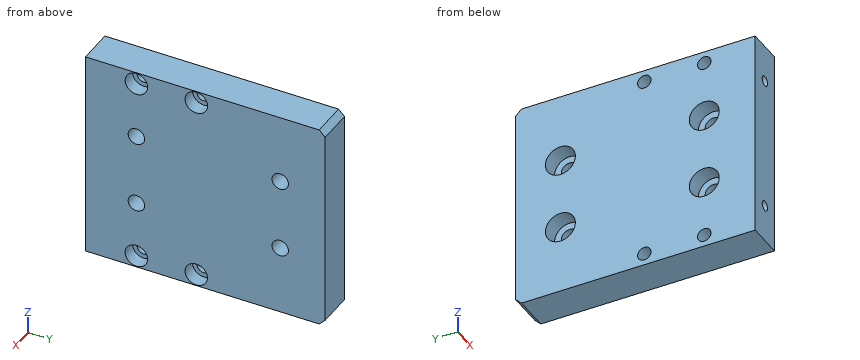
from build123d import *

# Parameters (mm, degrees)
SKETCH_1_W                   = 70
SKETCH_1_H                   = 80
EXTRUDE_1_DEPTH              = 12
HOLE_WIZARD_M5_1_D           = 5.5
HOLE_WIZARD_M5_1_CBORE_D     = 10
HOLE_WIZARD_M5_1_CBORE_DEPTH = 5.7
HOLE_WIZARD_M4_1_D           = 4.5
HOLE_WIZARD_M4_1_CBORE_D     = 7.5
HOLE_WIZARD_M4_1_CBORE_DEPTH = 4.6
HOLE_WIZARD_M4_1_2_D         = 3.3
HOLE_WIZARD_M4_1_2_DEPTH     = 10.1
HOLE_WIZARD_M4_1_2_TIP       = 0.991420021
CHAMFER_1_SIZE               = 2


with BuildPart() as part:
    # 草图1 → 凸台-拉伸1 (new body)
    with BuildSketch(Plane(origin=(0, 0, 0), x_dir=(0, 0, -1), z_dir=(1, 0, 0))):
        Rectangle(SKETCH_1_W, SKETCH_1_H)
    extrude(amount=EXTRUDE_1_DEPTH)

    # M5 六角圆柱头螺钉的柱形沉头孔1 (through all)
    with Locations(Plane.ZY):
        with Locations((-12, 25), (-12, -23), (12, -23), (12, 25)):
            CounterBoreHole(HOLE_WIZARD_M5_1_D / 2, HOLE_WIZARD_M5_1_CBORE_D / 2, HOLE_WIZARD_M5_1_CBORE_DEPTH)

    # Hole Wizard M4 _1 (through all)
    with Locations(Plane(origin=(12, 0, 0), x_dir=(0, 0, -1), z_dir=(1, 0, 0))):
        with Locations((-31, -23), (-31, -3), (31, -3), (31, -23)):
            CounterBoreHole(HOLE_WIZARD_M4_1_D / 2, HOLE_WIZARD_M4_1_CBORE_D / 2, HOLE_WIZARD_M4_1_CBORE_DEPTH)

    # Hole Wizard M4 _1 2
    with Locations(Plane(origin=(0, -40, 0), x_dir=(-1, 0, 0), z_dir=(0, -1, 0))):
        with Locations((-6, 22.5), (-6, -22.5)):
            Hole(HOLE_WIZARD_M4_1_2_D / 2, depth=HOLE_WIZARD_M4_1_2_DEPTH)
            with Locations((0, 0, -(HOLE_WIZARD_M4_1_2_DEPTH + HOLE_WIZARD_M4_1_2_TIP / 2))):  # 118° drill point
                Cone(0, HOLE_WIZARD_M4_1_2_D / 2, HOLE_WIZARD_M4_1_2_TIP, mode=Mode.SUBTRACT)

    # 倒角1
    chamfer_1_edges = [part.edges().sort_by_distance(p)[0] for p in [
        (6, 40, 35),
        (6, 40, -35),
    ]]
    chamfer(chamfer_1_edges, length=CHAMFER_1_SIZE)


solid = part.part
Geometry check sheet. Reference: the model listing, model coordinates, mm. Coordinates: 2 decimals unless noted, no trailing zeros. Write each loop counter-clockwise with the first axis right and the second up, starting at its lowest first coordinate (ties: lowest second). Pieces come first, ordered by that corner, then holes. Notation, with made-up numbers: (70, 69) -> (82, 69) arc R20 ccw to (82, 105) -> close; hole circle Ø8 at (22.5, 33.25). An arc over 180 degrees is marked (long way). One line per question, with ' | ' between items.
1. Depth check by flat-ended pin: pin 1 Ø8 at (y, z) = (27, 10.5) entering from -X; pin 2 Ø4 at (y, z) = (-21.5, 31.5) entering from +X; pin 3 Ø5 at (y, z) = (-21.5, -13) entering from -X. Enter the tip coordinate at first touch or a pass-through.
Answers:
pin 1: stops at x = 0 | pin 2: stops at x = 7.4 | pin 3: stops at x = 5.7
2. Cross-section at B-B on x = 2.25. State how many separate pieces and enclosed holes the cut face has, and give its area (3 significant figures).
Answers:
separate pieces: 1 | enclosed holes: 8 | area: 5,220 mm²
3. Cross-section at D-D on y = -31. Record the cut outline in (x, z).
Answers:
outline: (0, -35) -> (12, -35) -> (12, 35) -> (0, 35) -> close; hole circle Ø3.3 at (6, -22.5); hole circle Ø3.3 at (6, 22.5)
4. Cross-section at C-C on y = 25. Record the cut outline in (x, z).
Answers:
outline: (0, -35) -> (12, -35) -> (12, -14.75) -> (5.7, -14.75) -> (5.7, -17) -> (0, -17) -> close; (0, -7) -> (5.7, -7) -> (5.7, -9.25) -> (12, -9.25) -> (12, 9.25) -> (5.7, 9.25) -> (5.7, 7) -> (0, 7) -> close; (0, 17) -> (5.7, 17) -> (5.7, 14.75) -> (12, 14.75) -> (12, 35) -> (0, 35) -> close
5. Cross-section at A-A on z = -12. Record the cut outline in (x, y), and give its area (3 significant figures).
Answers:
outline: (0, -40) -> (12, -40) -> (12, -25.75) -> (5.7, -25.75) -> (5.7, -28) -> (0, -28) -> close; (0, -18) -> (5.7, -18) -> (5.7, -20.25) -> (12, -20.25) -> (12, 22.25) -> (5.7, 22.25) -> (5.7, 20) -> (0, 20) -> close; (0, 30) -> (5.7, 30) -> (5.7, 27.75) -> (12, 27.75) -> (12, 40) -> (0, 40) -> close | area: 777 mm²
6. Thickness scan on probe 1 along Y at (x, z) = (2.8, 12); probe 2 along Y at (x, z) = (10.25, 31); probe 3 along Z at (x, y) = (6, -37). Record the ranges inside material, lowest first. Write a range as from..to.
Answers:
probe 1: y = -40..-28, -18..20, 30..40 | probe 2: y = -40..-26.75, -19.25..-6.75, 0.75..40 | probe 3: z = -35..-24.15, -20.85..20.85, 24.15..35
